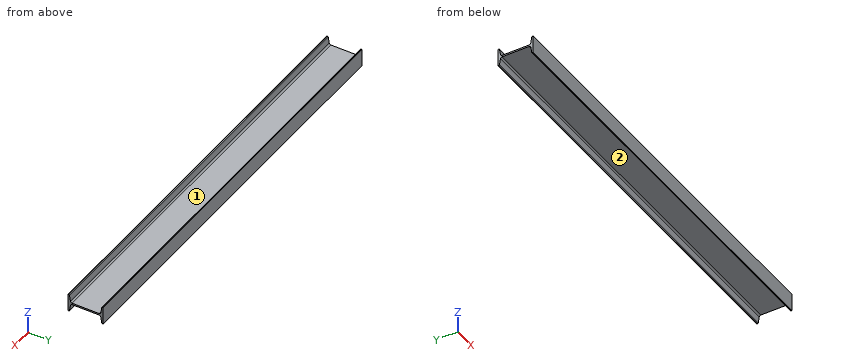
from build123d import *

# Parameters (mm, degrees)
BASE_DEPTH = 2400
FILLET1_R  = 9
FILLET2_R  = 4.5


with BuildPart() as part:
    # Sketch1 → Base (new body)
    with BuildSketch(Plane(origin=(0, 0, 0), x_dir=(0, 0, -1), z_dir=(1, 0, 0))):
        Polygon((-51, 0), (51, 0), (51, 6.775), (4.5, 14.525), (4.5, 185.475), (51, 193.225), (51, 200), (-51, 200), (-51, 193.225), (-4.5, 185.475), (-4.5, 14.525), (-51, 6.775), align=None)
    extrude(amount=BASE_DEPTH)

    # Fillet1
    fillet1_edges = [part.edges().sort_by_distance(p)[0] for p in [
        (1200, 14.525, 4.5),
        (1200, 185.475, 4.5),
        (1200, 185.475, -4.5),
        (1200, 14.525, -4.5),
    ]]
    fillet(fillet1_edges, radius=FILLET1_R)

    # Fillet2
    fillet2_edges = [part.edges().sort_by_distance(p)[0] for p in [
        (1200, 6.775, 51),
        (1200, 193.225, 51),
        (1200, 193.225, -51),
        (1200, 6.775, -51),
    ]]
    fillet(fillet2_edges, radius=FILLET2_R)


solid = part.part
Geometry check sheet. Reference: the model listing, model coordinates, mm. Face numbers are marked on the shaded views. A direction names the side the tool comes from. Coordinates: 2 decimals unless noted, no trailing zeros. Order: outer loops, then holes, each group sorted by start corner. A loop starts at its lowest first (then second) coordinate and runs counter-clockwise, first axis right, second up. Notation, with made-up numbers: (-14.5, 84.25) - (37.5, 84.25) arc R23 cw to (37.5, 109.25) - close; hole circle Ø8 at (47, -28.75). An arc over 180 degrees is marked (long way). One line per item, written item: value.
(1) Thickness scan on probe 1 along Z at (x, y) = (2092.5, 175); probe 2 along Y at (x, z) = (1357.5, -32); probe 3 along Y at (x, z) = (1869.5, -41). Record the ranges inside material, lowest first. Write a range as from..to.
Data:
probe 1: z = -4.5..4.5
probe 2: y = 0..9.94, 190.06..200
probe 3: y = 0..8.44, 191.56..200
(2) Sectioned sample at B-B (x = 1366). Enter the section's corners in (y, z).
Data:
outline: (0, -51) - (2.96, -51) arc R4.5 ccw to (7.4, -47.24) - (13.27, -12.02) arc R9 cw to (22.15, -4.5) - (177.85, -4.5) arc R9 cw to (186.73, -12.02) - (192.6, -47.24) arc R4.5 ccw to (197.04, -51) - (200, -51) - (200, 51) - (197.04, 51) arc R4.5 ccw to (192.6, 47.24) - (186.73, 12.02) arc R9 cw to (177.85, 4.5) - (22.15, 4.5) arc R9 cw to (13.27, 12.02) - (7.4, 47.24) arc R4.5 ccw to (2.96, 51) - (0, 51) - close
(3) Sectioned sample at A-A (z = 29.5). Enter the section's corners in (x, y).
Data:
outline: (0, 0) - (2400, 0) - (2400, 10.36) - (0, 10.36) - close; (0, 189.64) - (2400, 189.64) - (2400, 200) - (0, 200) - close
(4) Sectioned sample at C-C (y = 127). Enter the section's corners in (x, z).
Data:
outline: (0, -4.5) - (2400, -4.5) - (2400, 4.5) - (0, 4.5) - close
(5) Access from +Z, -Z, +X, -X, +Y, -Y to the whole of each face (thin tool, end or side, straight path). Record for the marked faces 1 and 2.
Data:
face 1: +Z, +X, -X
face 2: -Z, +X, -X
(6) Depth check by flat-ended pin: pin 1 Ø10 at (x, y) = (1144.5, 167) entering from -Z; pin 2 Ø12 at (x, y) = (888.5, 65) entering from +Z. Enter the tip coordinate at first touch or a pass-through.
Data:
pin 1: stops at z = -4.5
pin 2: stops at z = 4.5
